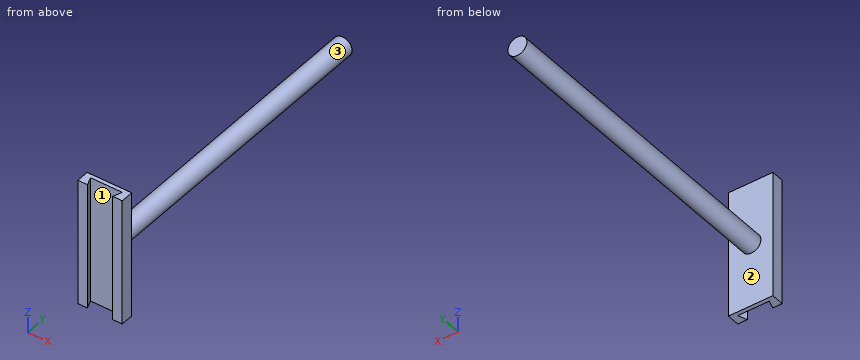
from build123d import *

# Parameters (mm, degrees)
BOSS_EXTRUDE1_DEPTH = 200
SKETCH2_R           = 15
BOSS_EXTRUDE2_DEPTH = 500


with BuildPart() as part:
    # Sketch1 → Boss-Extrude1 (new body)
    with BuildSketch(Plane.XY):
        Polygon((-30.262159038, 19.219105843), (39.737840962, 19.219105843), (39.737840962, -0.780894157), (24.737840962, -0.780894157), (29.737840962, 12.95649294), (-20.262159038, 12.95649294), (-15.262159038, -0.780894157), (-30.262159038, -0.780894157), align=None)
    extrude(amount=BOSS_EXTRUDE1_DEPTH)

    # Sketch2 → Boss-Extrude2 (add)
    with BuildSketch(Plane(origin=(0, 19.219105843, 0), x_dir=(1, 0, 0), z_dir=(0, 1, 0))):
        with Locations(Location((3.524411209, -100, 0), (0, 0, 90))):
            Circle(SKETCH2_R)
    extrude(amount=BOSS_EXTRUDE2_DEPTH)


solid = part.part
Here's how the part is built. I have some questions about the finished solid (model axes, mm). Face numbers are marked on the shaded views. Round coordinates to 2 decimals unless told otherwise and drop trailing zeros. Order: outer loops, then holes, each group sorted by start corner. A loop starts at its lowest first (then second) coordinate and runs counter-clockwise, first axis right, second up. Notation, with made-up numbers: M -5,-12.5 L 9,-12.5 A18 ccw 9,-3.5 Z; hole C 67.25,27 d8. An arc over 180 degrees is marked long. One line per question, with ' | ' between items.
1) Imagine slicing it at C-C, the plane z = 100. Write out the boundary of the cut face in (x, y).
Checked values:
outline: M -30.26,-0.78 L -15.26,-0.78 L -20.26,12.96 L 29.74,12.96 L 24.74,-0.78 L 39.74,-0.78 L 39.74,19.22 L 18.52,19.22 L 18.52,519.22 L -11.48,519.22 L -11.48,19.22 L -30.26,19.22 Z
2) I'm going to push flat-ended pins straight in: pin 1 Ø8 at (x, z) = (6, 167) entering from +Y; pin 2 Ø8 at (x, y) = (-3.5, 255.5) entering from -Z; pin 3 Ø15 at (x, z) = (0.5, 93.5) entering from -Y. Where does each tip first touch, or does it pass through?
Checked values:
pin 1: stops at y = 19.22 | pin 2: stops at z = 85.31 | pin 3: stops at y = 12.96
3) Imagine slicing it at D-D, the plane y = 99. Write out the boundary of the cut face in (x, z).
Checked values:
outline: C 3.52,100 d30
4) We'd pull the mould along Y, two halves only. Please class the marked faces 1, 2 and 3: released by +Y, released by -Y, zero draft, split by the parting line, or undercut.
Checked values:
face 1: undercut | face 2: released by +Y | face 3: zero draft
5) I need wall thicknesses on line 1 (Z direction, x = 4, y = 136); line 2 (Y direction, x = -12, z = 124.5); line 3 (Y direction, x = 33, z = 80.5). Which ranges of each line are inside material? Lowest first, please.
Checked values:
line 1: z = 85.01 to 114.99 | line 2: y = 12.96 to 19.22 | line 3: y = -0.78 to 19.22
6) Imagine slicing it at A-A, the plane z = 147.5. Write out the boundary of the cut face in (x, y), plus the area to 3 significant figures.
Checked values:
outline: M -30.26,-0.78 L -15.26,-0.78 L -20.26,12.96 L 29.74,12.96 L 24.74,-0.78 L 39.74,-0.78 L 39.74,19.22 L -30.26,19.22 Z | area: 782 mm²
7) Imagine slicing it at B-B, the plane x = 9. Write out the boundary of the cut face in (y, z), plus the area to 3 significant figures.
Checked values:
outline: M 12.96,0 L 19.22,0 L 19.22,86.04 L 519.22,86.04 L 519.22,113.96 L 19.22,113.96 L 19.22,200 L 12.96,200 Z | area: 15,200 mm²
